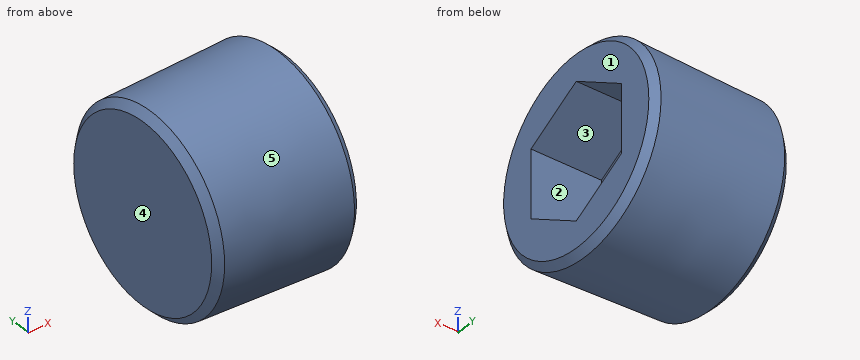
from build123d import *
from OCP.BRepFilletAPI import BRepFilletAPI_MakeChamfer

# Parameters (mm, degrees)
CUT_EXTRUDE_1_DEPTH = 5
CHAMFER_1_SIZE      = 0.5
CHAMFER_1_SIZE2     = 0.516477811
CHAMFER_1_SIZE2_2   = 0.485004947


with BuildPart() as part:
    # 草图1 → 旋转1 (revolve)
    with BuildSketch(Plane.XY):
        Polygon((0, 0), (0, 6.75), (10, 7.06426266), (10, 0), align=None)
    revolve(axis=Axis((0, 0, 0), (-1, 0, 0)))

    # 草图2 → 切除-拉伸1 (cut)
    with BuildSketch(Plane(origin=(10, 0, 0), x_dir=(0, 0, -1), z_dir=(1, 0, 0))):
        Polygon((2.367136104, -4.1), (4.734272207, 0), (2.367136104, 4.1), (-2.367136104, 4.1), (-4.734272207, 0), (-2.367136104, -4.1), align=None)
    extrude(amount=-CUT_EXTRUDE_1_DEPTH, mode=Mode.SUBTRACT)

    # 倒角1: one chamfer whose edges measure the first distance from different faces: ONE call of the kernel's chamfer builder (chamfer() names one face for all edges)
    chamfer_1_edges_1 = [part.edges().sort_by_distance(p)[0] for p in [
        (0, -6.75, 0),
    ]]
    chamfer_1_side_1 = [part.faces().sort_by_distance(p)[0] for p in [
        (0, 0, 0),
    ]]
    chamfer_1_edges_2 = [part.edges().sort_by_distance(p)[0] for p in [
        (10, -7.06426266, 0),
    ]]
    chamfer_1_side_2 = [part.faces().sort_by_distance(p)[0] for p in [
        (5, -6.90713133, 0),
    ]]
    chamfer_1 = BRepFilletAPI_MakeChamfer(part.part.solid().wrapped)
    for e in chamfer_1_edges_1:
        chamfer_1.Add(CHAMFER_1_SIZE, CHAMFER_1_SIZE2, e.wrapped, chamfer_1_side_1[0].wrapped)  # the first distance lies on this face
    for e in chamfer_1_edges_2:
        chamfer_1.Add(CHAMFER_1_SIZE, CHAMFER_1_SIZE2_2, e.wrapped, chamfer_1_side_2[0].wrapped)  # the first distance lies on this face
    add(Compound.cast(chamfer_1.Shape()), mode=Mode.REPLACE)


solid = part.part
The model under review builds one solid part; all positions refer to its coordinate system, in mm. Face numbers are marked on the shaded views. A direction names the side the tool comes from. Round coordinates to 2 decimals unless told otherwise and drop trailing zeros. Order: outer loops, then holes, each group sorted by start corner. A loop starts at its lowest first (then second) coordinate and runs counter-clockwise, first axis right, second up. Notation, with made-up numbers: (-5.75, 41.5) - (42.25, 41.5) arc R33 ccw to (42.25, 69.5) - close; hole circle Ø6 at (-39, -9.5). An arc over 180 degrees is marked (long way). Use one line per item in the form item = value.
Q1. Add section A-A on x = 6.5. Give the boundary of the cut face in (y, z).
Response values:
outline = circle Ø13.91 at (0, 0); hole (-4.1, -2.37) - (0, -4.73) - (4.1, -2.37) - (4.1, 2.37) - (0, 4.73) - (-4.1, 2.37) - close
Q2. Mouldability with a two-part tool opening along Y and no side actions: class the marked faces 3, 4 and 5 as pulls with the +Y half, pulls with the -Y half, needs draft (parallel to the pull), parting line crosses it, or undercut.
Response values:
face_3 = undercut
face_4 = needs draft
face_5 = parting line crosses it
Q3. Add section D-D on x = 2. Give the boundary of the cut face in (y, z), then the cut area to 3 significant figures.
Response values:
outline = circle Ø13.63 at (0, 0)
area = 146 mm^2
Q4. Add section C-C on x = 8.25. Give the boundary of the cut face in (y, z).
Response values:
outline = circle Ø14.02 at (0, 0); hole (-4.1, -2.37) - (0, -4.73) - (4.1, -2.37) - (4.1, 2.37) - (0, 4.73) - (-4.1, 2.37) - close
Q5. To check wall thickness, follow line 1 (Z direction, x = 5.5, y = -1.5); line 2 (Y direction, x = 9.25, z = 1); line 3 (Z direction, x = 6.25, y = 2.75). State the ranges of each line that lie inside material, in increasing order.
Response values:
line_1 = -6.76 to -3.87, 3.87 to 6.76
line_2 = -6.97 to -4.1, 4.1 to 6.97
line_3 = -6.38 to -3.15, 3.15 to 6.38
Q6. Add section B-B on z = 0. Give the boundary of the cut face in (x, y), then the cut area to 3 significant figures.
Response values:
outline = (0, -6.25) - (0.52, -6.77) - (9.5, -7.05) - (10, -6.58) - (10, -4.1) - (5, -4.1) - (5, 4.1) - (10, 4.1) - (10, 6.58) - (9.5, 7.05) - (0.52, 6.77) - (0, 6.25) - close
area = 96.6 mm^2
Q7. Tool access review of the marked faces 1 and 2: name each direction out of +Z, -Z, +X, -X, +Y, -Y from which nothing blocks a thin tool from reaching the whole face with its end or side.
Response values:
face_1 = +Z, -Z, +X, +Y, -Y
face_2 = +X
Q8. Clearance check with flat-ended pins moving along their axes: P1, Ø1, axis at x = 5, z = -2.5, coming from the +Y side; P2, Ø4, axis at x = 7.5, y = -0.5, coming from the -Z side; P3, Ø1.5, axis at x = 6, y = -4.5, coming from the +Z side. State where each tip first meets the part, or that it passes through.
Response values:
P1 = 6.61
P2 = -7.05
P3 = 5.84
